Geometry check sheet. Reference: the model listing, model coordinates, mm. Face numbers are marked on the shaded views. Round coordinates to 2 decimals unless told otherwise and drop trailing zeros. Loops run counter-clockwise (first coordinate to the right, second up) from the corner with the lowest first, then second, coordinate; pieces in that order, holes last. Notation, with made-up numbers: (-21, 87) - (34, 87) arc R28 cw to (34, 120) - close; hole circle Ø5 at (-12, 51.25). An arc over 180 degrees is marked (long way). Write item = value, one per line.
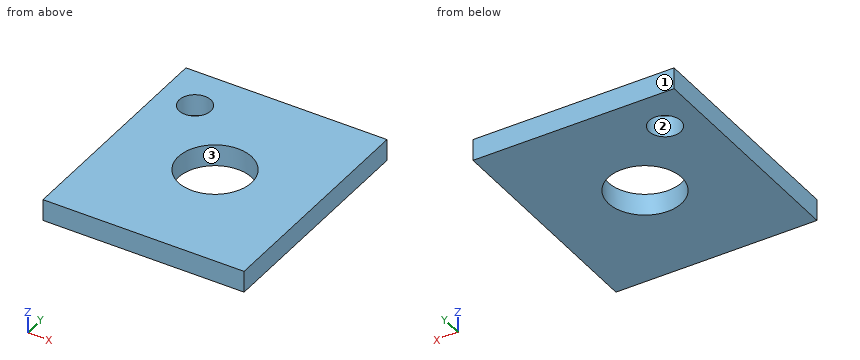
```python
from build123d import *

# Parameters (mm, degrees)
SKETCH_1_W          = 28
SKETCH_1_H          = 32
EXTRUDE_1_DEPTH     = 1.5
SKETCH_2_R          = 5.1
SKETCH_2_R_2        = 2.2
CUT_EXTRUDE_1_DEPTH = 11.5


with BuildPart() as part:
    # 草图1 → 凸台-拉伸1 (new, symmetric)
    with BuildSketch(Plane.XY):
        Rectangle(SKETCH_1_W, SKETCH_1_H)
    extrude(amount=EXTRUDE_1_DEPTH, both=True)

    # 草图2 → 切除-拉伸1 (cut, symmetric)
    with BuildSketch(Plane.XY):
        Circle(SKETCH_2_R)
        with Locations((-9, 10)):
            Circle(SKETCH_2_R_2)
    extrude(amount=CUT_EXTRUDE_1_DEPTH, both=True, mode=Mode.SUBTRACT)


solid = part.part
```
(1) Section check A-A (y = 10). Enter the section's corners in (x, z), then the cut area to 3 significant figures.
Answers follow:
outline = (-14, -1.5) - (-11.2, -1.5) - (-11.2, 1.5) - (-14, 1.5) - close; (-6.8, -1.5) - (14, -1.5) - (14, 1.5) - (-6.8, 1.5) - close
area = 70.8 mm²
(2) Section check C-C (z = 0.05). Enter the section's corners in (x, y).
Answers follow:
outline = (-14, -16) - (14, -16) - (14, 16) - (-14, 16) - close; hole circle Ø4.4 at (-9, 10); hole circle Ø10.2 at (0, 0)
(3) Mould release check, pull along X, two halves, no side actions. Record for the marked faces 1, 2 and 3: pulls with the +X half, pulls with the -X half, needs draft (parallel to the pull), parting line crosses it, or undercut.
Answers follow:
face_1 = needs draft
face_2 = undercut
face_3 = undercut
(4) Scan lines: L1, parallel to Y at x = 0, z = 0.45; L2, parallel to Y at x = -9, z = -0.65; L3, parallel to X at y = 0, z = 0.3. Record each from-to range of solid material in increasing order. Write a range as [from, to].
Answers follow:
L1 = [-16, -5.1], [5.1, 16]
L2 = [-16, 7.8], [12.2, 16]
L3 = [-14, -5.1], [5.1, 14]
(5) Section check B-B (x = 0). Enter the section's corners in (y, z), then the cut area to 3 significant figures.
Answers follow:
outline = (-16, -1.5) - (-5.1, -1.5) - (-5.1, 1.5) - (-16, 1.5) - close; (5.1, -1.5) - (16, -1.5) - (16, 1.5) - (5.1, 1.5) - close
area = 65.4 mm²
